Part model, mm, in its own coordinate system. Round coordinates to 2 decimals unless told otherwise and drop trailing zeros. Loops run counter-clockwise (first coordinate to the right, second up) from the corner with the lowest first, then second, coordinate; pieces in that order, holes last. Notation, with made-up numbers: M 28.5,61.25 L 71.5,61.25 A31 cw 71.5,99.25 Z; hole C 18.25,56 d5. An arc over 180 degrees is marked long. Put each result on its own line as item: value. Start each with the question number.
1) Slice it at C-C on y = 34. Give the cut face in (x, z).
2) Slice it at A-A on z = 5.5. Give the cut face in (x, y), then the cut area to 3 significant figures.
3) Slice it at B-B on x = 75. Give the cut face in (y, z), then the cut area to 3 significant figures.
4) Probe line 1 along Y through (x, z) = (75, 18.5); line 2 along Y through (x, z) = (81.5, 17.5); line 3 along X through (y, z) = (113.5, 7). List the from-to ranges inside material, lowest first.
5) Pull direction Y, two halves, no side cores. Call faces 1 (the flat face through (59, 120, 12)), 2 (the cylindrical face through (5.703, 6.014, 12.675)), 3 (the flat face through (59, 61, 25)), 4 (the cylindrical face through (67, 34, 12)): +Y half, -Y half, draft (parallel to the pull), parting line (faces both ways), or undercut.
```python
from build123d import *

# Parameters (mm, degrees)
SKETCH1_W           = 120
SKETCH1_H           = 120
SKETCH1_R           = 10
BOSS_EXTRUDE1_DEPTH = 25
FILLET1_R           = 20


with BuildPart() as part:
    # Sketch1 → Boss-Extrude1 (new body)
    with BuildSketch(Plane.XY):
        with Locations((60, 60)):
            Rectangle(SKETCH1_W, SKETCH1_H)
        with Locations((75, 40)):
            Circle(SKETCH1_R, mode=Mode.SUBTRACT)
    extrude(amount=BOSS_EXTRUDE1_DEPTH)

    # Fillet1
    fillet1_edges = [part.edges().sort_by_distance(p)[0] for p in [
        (0, 120, 12.5),
        (120, 120, 12.5),
        (120, 0, 12.5),
        (0, 0, 12.5),
    ]]
    fillet(fillet1_edges, radius=FILLET1_R)


solid = part.part
```
Recorded:
1. outline: M 0,0 L 67,0 L 67,25 L 0,25 Z; M 83,0 L 120,0 L 120,25 L 83,25 Z
2. outline: M 0,20 A20 ccw 20,0 L 100,0 A20 ccw 120,20 L 120,100 A20 ccw 100,120 L 20,120 A20 ccw 0,100 Z; hole C 75,40 d20
2. area: 13,700 mm2
3. outline: M 0,0 L 30,0 L 30,25 L 0,25 Z; M 50,0 L 120,0 L 120,25 L 50,25 Z
3. area: 2,500 mm2
4. line 1: y = 0 to 30, 50 to 120
4. line 2: y = 0 to 32.4, 47.6 to 120
4. line 3: x = 5.24 to 114.76
5. face 1: +Y half
5. face 2: -Y half
5. face 3: draft
5. face 4: undercut
